Design review of the part shown in the three views and the two pictorial views. Dimensions are in mm from the part's minimum x, y and z. A direction names the side the tool comes from. Give positions to 0.01 mm unless a question says otherwise; leave off trailing zeros. Loops run counter-clockwise (first coordinate to the right, second up) from the corner with the lowest first, then second, coordinate; pieces in that order, holes last. Notation, with made-up numbers: (73.25, -12) - (130.25, -12) arc R34 ccw to (130.25, 22) - close; hole circle Ø1 at (-12.5, -24.5). An arc over 180 degrees is marked (long way). Return JSON: item names as keys, results as strings. Group by question number.
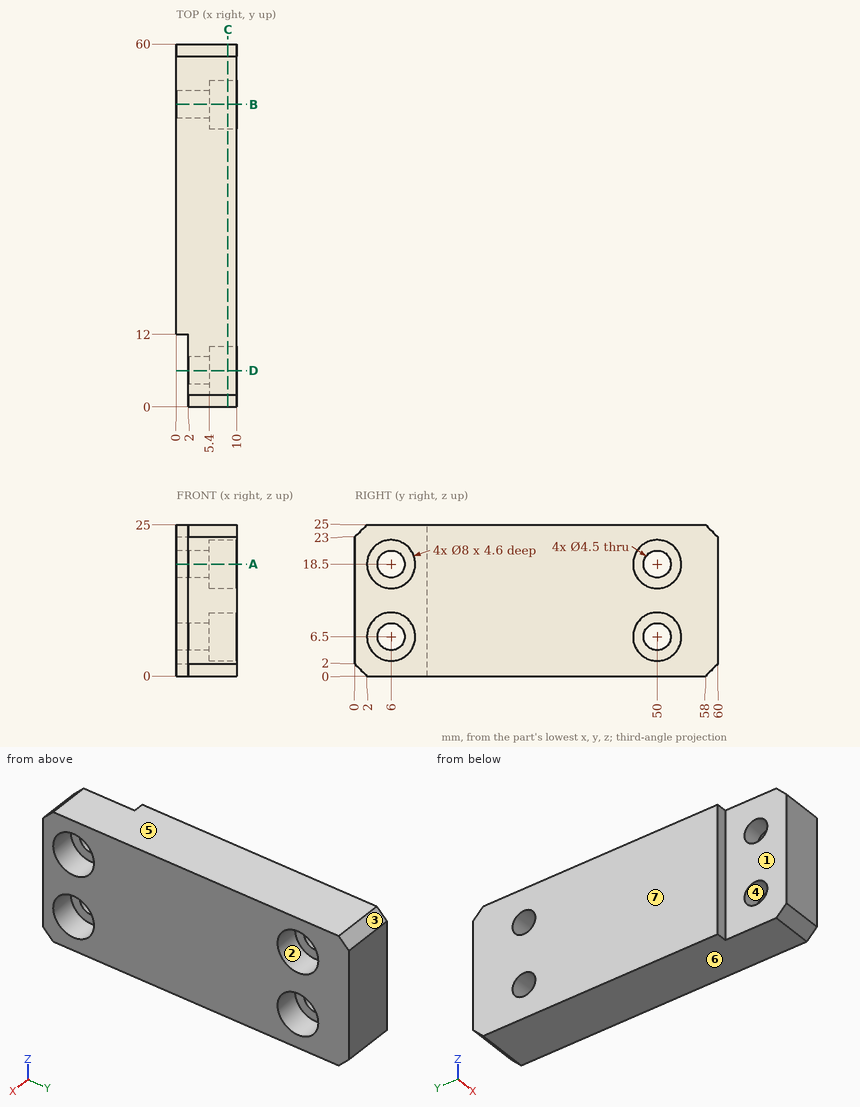
Item 1: Tool access review of the marked faces 1, 2 and 3: name each direction out of +Z, -Z, +X, -X, +Y, -Y from which nothing blocks a thin tool from reaching the whole face with its end or side.
Item 2: Take a section at A-A (z = 18.5). State the section outline as (x, y) points.
Item 3: Take a section at B-B (y = 50). State the section outline as (x, z) points, then the cut area to 3 significant figures.
Item 4: For L1, parallel to Y at x = 2.35, z = 18.5; L2, parallel to Y at x = 8.3, z = 18.5; L3, parallel to Z at x = 0.5, y = 51, list the stretches that pass through material, from the lowest coordinate up. Write a range as from..to.
Item 5: Take a section at C-C (x = 8.5). State the section outline as (y, z) points, then the cut area to 3 significant figures.
Item 6: Mouldability with a two-part tool opening along Z and no side actions: class the marked faces 4, 5, 6 and 7 as +Z half, -Z half, draft (parallel to the pull), parting line (faces both ways), or undercut.
Item 7: For P1, Ø3.5, axis at y = 50, z = 18.5, coming from the +X side; P2, Ø1.6, axis at x = 1, z = 10.5, coming from the -Y side; P3, Ø5, axis at y = 50, z = 6.5, coming from the +X side, all flat-tipped, find the tip position at first contact; note any pin that passes through.
Item 8: Take a section at D-D (y = 6). State the section outline as (x, z) points.
Check sheet entries:
{
 "1": {"face 1": "+Z, -Z, -X, -Y", "face 2": "+X", "face 3": "+Z, +X, -X, +Y"},
 "2": {"outline": "(0, 12) - (2, 12) - (2, 8.25) - (5.4, 8.25) - (5.4, 10) - (10, 10) - (10, 46) - (5.4, 46) - (5.4, 47.75) - (0, 47.75) - close; (0, 52.25) - (5.4, 52.25) - (5.4, 54) - (10, 54) - (10, 60) - (0, 60) - close; (2, 0) - (10, 0) - (10, 2) - (5.4, 2) - (5.4, 3.75) - (2, 3.75) - close"},
 "3": {"outline": "(0, 0) - (10, 0) - (10, 2.5) - (5.4, 2.5) - (5.4, 4.25) - (0, 4.25) - close; (0, 8.75) - (5.4, 8.75) - (5.4, 10.5) - (10, 10.5) - (10, 14.5) - (5.4, 14.5) - (5.4, 16.25) - (0, 16.25) - close; (0, 20.75) - (5.4, 20.75) - (5.4, 22.5) - (10, 22.5) - (10, 25) - (0, 25) - close", "area": "128 mm^2"},
 "4": {"L1": "y = 0..3.75, 8.25..47.75, 52.25..60", "L2": "y = 0..2, 10..46, 54..60", "L3": "z = 0..4.48, 8.52..16.48, 20.52..25"},
 "5": {"outline": "(0, 2) - (2, 0) - (58, 0) - (60, 2) - (60, 23) - (58, 25) - (2, 25) - (0, 23) - close; hole circle Ø8 at (6, 6.5); hole circle Ø8 at (6, 18.5); hole circle Ø8 at (50, 6.5); hole circle Ø8 at (50, 18.5)", "area": "1,290 mm^2"},
 "6": {"face 4": "undercut", "face 5": "+Z half", "face 6": "-Z half", "face 7": "draft"},
 "7": {"P1": "passes through", "P2": "stops at y = 12", "P3": "stops at x = 5.4"},
 "8": {"outline": "(2, 0) - (10, 0) - (10, 2.5) - (5.4, 2.5) - (5.4, 4.25) - (2, 4.25) - close; (2, 8.75) - (5.4, 8.75) - (5.4, 10.5) - (10, 10.5) - (10, 14.5) - (5.4, 14.5) - (5.4, 16.25) - (2, 16.25) - close; (2, 20.75) - (5.4, 20.75) - (5.4, 22.5) - (10, 22.5) - (10, 25) - (2, 25) - close"}
}
